from build123d import *

# Parameters (mm, degrees)
SKETCH1_W           = 236.3
SKETCH1_H           = 194
BOSS_EXTRUDE1_DEPTH = 6
CUT_EXTRUDE1_DEPTH  = 2
CUT_EXTRUDE2_DEPTH  = 154.194068097
FILLET1_R           = 5
SKETCH4_R           = 2
CUT_EXTRUDE3_DEPTH  = 2
SKETCH5_R           = 1.5
CUT_EXTRUDE4_DEPTH  = 4
SKETCH7_R           = 2
CUT_EXTRUDE6_DEPTH  = 4
SKETCH8_R           = 2
CUT_EXTRUDE7_DEPTH  = 4


with BuildPart() as part:
    # Sketch1 → Boss-Extrude1 (new, symmetric)
    with BuildSketch(Plane.XY):
        Rectangle(SKETCH1_W, SKETCH1_H)
    extrude(amount=BOSS_EXTRUDE1_DEPTH, both=True)

    # Sketch2 → Cut-Extrude1 (cut)
    with BuildSketch(Plane.XY.offset(6)):
        Polygon((108.15, 87), (-108.15, 87), (-108.15, -87), (93.15, -87), (93.15, -62), (108.15, -62), align=None)
    extrude(amount=-CUT_EXTRUDE1_DEPTH, mode=Mode.SUBTRACT)

    # Sketch3 → Cut-Extrude2 (cut, through all)
    with BuildSketch(Plane.XY.offset(4)):
        Polygon((90.15, -84), (90.15, -59), (105.15, -59), (105.15, 84), (-105.15, 84), (-105.15, -84), align=None)
    extrude(amount=-CUT_EXTRUDE2_DEPTH, mode=Mode.SUBTRACT)

    # Fillet1
    fillet1_edges = [part.edges().sort_by_distance(p)[0] for p in [
        (90.15, -84, -1),
        (-105.15, -84, -1),
        (-105.15, 84, -1),
        (105.15, 84, -1),
    ]]
    fillet(fillet1_edges, radius=FILLET1_R)

    # Sketch4 → Cut-Extrude3 (cut)
    with BuildSketch(Plane.ZY.offset(118.15)):
        with Locations(Location((0, 0, 0), (0, 0, 270))):
            Circle(SKETCH4_R)
        with Locations(Location((0, 70, 0), (0, 0, 270))):
            Circle(SKETCH4_R)
        with Locations(Location((0, -70, 0), (0, 0, 90))):
            Circle(SKETCH4_R)
    cut_extrude3 = extrude(amount=-CUT_EXTRUDE3_DEPTH, mode=Mode.SUBTRACT)

    # Mirror1: Cut-Extrude3 across plane
    add(cut_extrude3.mirror(Plane(origin=(0, 0, 0), x_dir=(0, 0, 1), z_dir=(1, 0, 0))), mode=Mode.SUBTRACT)

    # Sketch5 → Cut-Extrude4 (cut)
    with BuildSketch(Plane(origin=(0, 97, 0), x_dir=(1, 0, 0), z_dir=(0, 1, 0))):
        with Locations(Location((-90, 0, 0), (0, 0, 270))):
            Circle(SKETCH5_R)
        with Locations(Location((90, 0, 0), (0, 0, 90))):
            Circle(SKETCH5_R)
    cut_extrude4 = extrude(amount=-CUT_EXTRUDE4_DEPTH, mode=Mode.SUBTRACT)

    # Mirror2: Cut-Extrude4 across plane
    add(cut_extrude4.mirror(Plane.ZX), mode=Mode.SUBTRACT)

    # Sketch7 → Cut-Extrude6 (cut)
    with BuildSketch(Plane.XY.offset(6)):
        with Locations((-113.15, 78)):
            Circle(SKETCH7_R)
        with Locations((-113.15, 28)):
            Circle(SKETCH7_R)
        with Locations((-113.15, -22)):
            Circle(SKETCH7_R)
        with Locations((-113.15, -42)):
            Circle(SKETCH7_R)
        with Locations((-113.15, -62)):
            Circle(SKETCH7_R)
    cut_extrude6 = extrude(amount=-CUT_EXTRUDE6_DEPTH, mode=Mode.SUBTRACT)

    # Mirror3: Cut-Extrude6 across plane
    add(cut_extrude6.mirror(Plane(origin=(0, 0, 0), x_dir=(0, 0, 1), z_dir=(1, 0, 0))), mode=Mode.SUBTRACT)

    # Sketch8 → Cut-Extrude7 (cut)
    with BuildSketch(Plane.XY.offset(6)):
        with Locations((0, 92)):
            Circle(SKETCH8_R)
    extrude(amount=-CUT_EXTRUDE7_DEPTH, mode=Mode.SUBTRACT)


solid = part.part
Part model, mm, in its own coordinate system. A direction names the side the tool comes from. Round coordinates to 2 decimals unless told otherwise and drop trailing zeros. Write each loop counter-clockwise with the first axis right and the second up, starting at its lowest first coordinate (ties: lowest second). Pieces come first, ordered by that corner, then holes. Notation, with made-up numbers: M 59,-25 L 77,-25 A28 cw 77,6 Z; hole C -30.75,73 d10. An arc over 180 degrees is marked long. Return JSON: item names as keys, results as strings. Group by question number.
(1) Which spindle directions (+Z, -Z, +X, -X, +Y, -Y) get a long thin tool onto all of the face, cutting with end or side? Do faces 1 (the face through (103.72, 82.5, -1.07)), 2 (the face through (8, -93, 6)). Say none if no direction does.
(2) Pin check, flat tips, straight feed: pin 1 Ø3.5 at (y, z) = (0, 0) entering from +X; pin 2 Ø3.5 at (x, y) = (113.15, -22) entering from +Z; pin 3 Ø1.8 at (x, z) = (-90, 0) entering from -Y. Stop position of each tip, or through.
(3) Saw through at A-A on y = 10.5. Write the cut outline in (x, z), then the cut area to 3 significant figures.
(4) Drill centre lines: probe 1 along Y at (x, z) = (113.15, 3.3); probe 2 along Y at (x, z) = (0, 3.95); probe 3 along X at (y, z) = (93.9, 0). Where is each one in solid material? Low to high.
(5) Saw through at B-B on x = 63. Write the cut outline in (y, z).
(6) Two-plate mould, pull along Y, no slides. Class faces 3 (the face through (90.15, -69, -1)), 4 (the face through (-2, 97, 0)), 5 (the face through (-2, -97, 0)): +Y half, -Y half, draft (parallel to the pull), parting line (faces both ways), or undercut.
Returned:
{
 "1": {"face 1": "+Z, -Z", "face 2": "+Z, +X, -X, +Y, -Y"},
 "2": {"pin 1": "x = 116.15", "pin 2": "z = 2", "pin 3": "y = -93"},
 "3": {"outline": "M -118.15,-6 L -105.15,-6 L -105.15,4 L -108.15,4 L -108.15,6 L -118.15,6 Z; M 105.15,-6 L 118.15,-6 L 118.15,6 L 108.15,6 L 108.15,4 L 105.15,4 Z", "area": "300 mm²"},
 "4": {"probe 1": "-97 to -64, -60 to -44, -40 to -24, -20 to 26, 30 to 76, 80 to 97", "probe 2": "-97 to -84, 84 to 90, 94 to 97", "probe 3": "-118.15 to -91.5, -88.5 to 88.5, 91.5 to 118.15"},
 "5": {"outline": "M -97,-6 L -84,-6 L -84,4 L -87,4 L -87,6 L -97,6 Z; M 84,-6 L 97,-6 L 97,6 L 87,6 L 87,4 L 84,4 Z"},
 "6": {"face 3": "undercut", "face 4": "+Y half", "face 5": "-Y half"}
}
